```python
from build123d import *

# Parameters (mm, degrees)
SKETCH1_R           = 7
BOSS_EXTRUDE1_DEPTH = 3
SKETCH2_R           = 4.5
BOSS_EXTRUDE2_DEPTH = 30
CHAMFER1_SIZE       = 1
CHAMFER2_SIZE       = 0.5


with BuildPart() as part:
    # Sketch1 → Boss-Extrude1 (new body)
    with BuildSketch(Plane(origin=(0, 0, 0), x_dir=(1, 0, 0), z_dir=(0, 1, 0))):
        with Locations(Location((0, 0, 0), (0, 0, 270))):
            Circle(SKETCH1_R)
    extrude(amount=BOSS_EXTRUDE1_DEPTH)

    # Sketch2 → Boss-Extrude2 (add)
    with BuildSketch(Plane(origin=(0, 3, 0), x_dir=(1, 0, 0), z_dir=(0, 1, 0))):
        with Locations(Location((0, 0, 0), (0, 0, 270))):
            Circle(SKETCH2_R)
    extrude(amount=BOSS_EXTRUDE2_DEPTH)

    # Chamfer1
    chamfer1_edges = [part.edges().sort_by_distance(p)[0] for p in [
        (0, 33, -4.5),
    ]]
    chamfer(chamfer1_edges, length=CHAMFER1_SIZE)

    # Chamfer2
    chamfer2_edges = [part.edges().sort_by_distance(p)[0] for p in [
        (0, 0, -7),
        (0, 3, -7),
    ]]
    chamfer(chamfer2_edges, length=CHAMFER2_SIZE)


solid = part.part
```
Check sheet for the modelled part. Datum: model origin and axes. Units: mm. Give positions to 0.01 mm unless a question says otherwise; leave off trailing zeros. Order: outer loops, then holes, each group sorted by start corner. A loop starts at its lowest first (then second) coordinate and runs counter-clockwise, first axis right, second up. Notation, with made-up numbers: M 38,73 L 72,73 A23 cw 72,86 Z; hole C 2.5,-14 d4. An arc over 180 degrees is marked long. Answer in a Markdown table with one row per item. Add a question column.
Q1. Sectioned sample at B-B, the plane z = 0. Record the boundary of the cut face in (x, y).
Q2. Gauge pin test, flat ends, axial feed: pin 1 Ø3 at (y, z) = (8, 2) entering from -X; pin 2 Ø1 at (x, y) = (-2.5, 7) entering from +Z; pin 3 Ø4 at (x, y) = (1.5, 17) entering from +Z. Record the tip position at first contact, or that the pin passes through.
Q3. Sectioned sample at A-A, the plane x = 0. Record the boundary of the cut face in (y, z).
Q4. Sectioned sample at C-C, the plane y = 20.5. Record the boundary of the cut face in (x, z), and give its area (3 significant figures).
Q5. Release check for a two-part mould opening along Y. For faces 1 (the flat face through (0, 33, 0)), 2 (the cylindrical face through (-6.834, 1.486, -1.517)), 3 (the flat face through (0, 0, 0)) record: released by +Y, released by -Y, zero draft, split by the parting line, or undercut.
Q6. Thickness scan on L1, parallel to Y at x = 3.25, z = 3.5; L2, parallel to X at y = 8.5, z = -2.5; L3, parallel to Z at x = -3, y = 6. Record the ranges inside material, lowest first.
Verdict:
| question | item | result |
|---|---|---|
| 1 | outline | M -7,0.5 L -6.5,0 L 6.5,0 L 7,0.5 L 7,2.5 L 6.5,3 L 4.5,3 L 4.5,32 L 3.5,33 L -3.5,33 L -4.5,32 L -4.5,3 L -6.5,3 L -7,2.5 Z |
| 2 | pin 1 | x = -4.47 |
| 2 | pin 2 | z = 4.03 |
| 2 | pin 3 | z = 4.5 |
| 3 | outline | M 0,-6.5 L 0.5,-7 L 2.5,-7 L 3,-6.5 L 3,-4.5 L 32,-4.5 L 33,-3.5 L 33,3.5 L 32,4.5 L 3,4.5 L 3,6.5 L 2.5,7 L 0.5,7 L 0,6.5 Z |
| 4 | outline | C 0,0 d9 |
| 4 | area | 63.6 mm² |
| 5 | face 1 | released by +Y |
| 5 | face 2 | zero draft |
| 5 | face 3 | released by -Y |
| 6 | L1 | 0 to 3 |
| 6 | L2 | -3.74 to 3.74 |
| 6 | L3 | -3.35 to 3.35 |
